```python
from build123d import *

# Parameters (mm, degrees)
SKETCH_1_W               = 1204
SKETCH_1_H               = 210
EXTRUDE_1_DEPTH          = 30
SHELL_1_T                = -2
SKETCH_2_W               = 1204
SKETCH_2_H               = 20
EXTRUDE_2_DEPTH          = 2
CUT_EXTRUDE_1_DEPTH      = 1477
CUT_EXTRUDE_1_DEPTH_BACK = 116
SKETCH_3_R               = 4.5
SKETCH_4_R               = 4.5
CUT_EXTRUDE_2_DEPTH      = 116


with BuildPart() as part:
    # 草图1 → 凸台-拉伸1 (new body)
    with BuildSketch(Plane.XY):
        with Locations((602, 105)):
            Rectangle(SKETCH_1_W, SKETCH_1_H)
    extrude(amount=EXTRUDE_1_DEPTH)

    # 抽壳1
    shell_1_openings = [part.faces().sort_by_distance(p)[0] for p in [
        (602, 105, 30),
    ]]
    offset(amount=SHELL_1_T, openings=shell_1_openings, kind=Kind.INTERSECTION)

    # 草图2 → 凸台-拉伸2 (add)
    with BuildSketch(Plane.XY.offset(30)):
        with Locations((602, 220)):
            Rectangle(SKETCH_2_W, SKETCH_2_H)
    extrude(amount=-EXTRUDE_2_DEPTH)

    # 草图3 → 切除-拉伸1 (cut, two sides: drawn at the far end of the back side and taken through both)
    with BuildSketch(Plane(origin=(2, 0, 0), x_dir=(0, 0, -1), z_dir=(1, 0, 0)).offset(-CUT_EXTRUDE_1_DEPTH_BACK)):
        with Locations(Location((-16, 180, 0), (0, 0, 180))):
            Circle(SKETCH_3_R)
        with Locations(Location((-16, 30, 0), (0, 0, 180))):
            Circle(SKETCH_3_R)
    extrude(amount=CUT_EXTRUDE_1_DEPTH + CUT_EXTRUDE_1_DEPTH_BACK, mode=Mode.SUBTRACT)

    # 草图4 → 切除-拉伸2 (cut)
    with BuildSketch(Plane(origin=(0, 2, 0), x_dir=(1, 0, 0), z_dir=(0, 1, 0))):
        with Locations(Location((30, -16, 0), (0, 0, 270))):
            Circle(SKETCH_4_R)
        with Locations(Location((1174, -16, 0), (0, 0, 270))):
            Circle(SKETCH_4_R)
        with Locations(Location((602, -16, 0), (0, 0, 270))):
            Circle(SKETCH_4_R)
    extrude(amount=-CUT_EXTRUDE_2_DEPTH, mode=Mode.SUBTRACT)


solid = part.part
```
Model file for the job. Use its own axes, mm. A direction names the side the tool comes from. Round coordinates to 2 decimals unless told otherwise and drop trailing zeros. Write each loop counter-clockwise with the first axis right and the second up, starting at its lowest first coordinate (ties: lowest second). Pieces come first, ordered by that corner, then holes. Notation, with made-up numbers: M 52.5,-21 L 83.5,-21 A32 cw 83.5,15 Z; hole C -40,13 d6. An arc over 180 degrees is marked long. Put each result on its own line as item: value.
Item 1: Tool access for faces 5 (the flat face through (594, 106, 0)), 6 (the flat face through (1202, 104, 16)), 7 (the flat face through (594, 220, 28)): list every direction of +Z, -Z, +X, -X, +Y, -Y with a clear straight run to the whole face (end or side of a thin tool).
Responses:
face 5: -Z, +X, -X, +Y, -Y
face 6: +Z
face 7: -Z, +X, -X, +Y
Item 2: Probe L1, parallel to Y at x = 1202.75, z = 16; L2, parallel to X at y = 65.5, z = 3; L3, parallel to X at y = 0.75, z = 16. List the from-to ranges inside material, lowest first. Write a range as from..to.
Responses:
L1: 0..25.5, 34.5..175.5, 184.5..210
L2: 0..2, 1202..1204
L3: 0..25.5, 34.5..597.5, 606.5..1169.5, 1178.5..1204
Item 3: Flat gauge pins, fed straight in: P1, Ø14.5, axis at x = 30, z = 16, coming from the +Y side; P2, Ø8, axis at y = 180, z = 16, coming from the -X side; P3, Ø22, axis at x = 615, y = 223.5, coming from the -Z side; P4, Ø10, axis at x = 558.5, y = 108, coming from the +Z side. Where does each tip first touch, or does it go through?
Responses:
P1: y = 210
P2: through
P3: z = 28
P4: z = 2
Item 4: Mould opens along Y. For faces 1 (the flat face through (594, 0, 15)), 2 (the flat face through (1204, 113, 15)), 3 (the flat face through (594, 2, 16)), 4 (the flat face through (594, 106, 2)) say: +Y half, -Y half, draft (parallel to the pull), parting line (faces both ways), or undercut.
Responses:
face 1: -Y half
face 2: draft
face 3: undercut
face 4: undercut
Item 5: Cut at A-A (x = 438). List the corners of the cut face in (y, z), and give its area (3 significant figures).
Responses:
outline: M 0,0 L 210,0 L 210,28 L 230,28 L 230,30 L 208,30 L 208,2 L 2,2 L 2,30 L 0,30 Z
area: 572 mm²
Item 6: Cut at B-B (y = 55). List the corners of the cut face in (x, z), and give its area (3 significant figures).
Responses:
outline: M 0,0 L 1204,0 L 1204,30 L 1202,30 L 1202,2 L 2,2 L 2,30 L 0,30 Z
area: 2,520 mm²
Item 7: Cut at C-C (z = 16). State how many separate pieces and enclosed holes the cut face has, and give its area (3 significant figures).
Responses:
separate pieces: 7
enclosed holes: 0
area: 5,510 mm²
